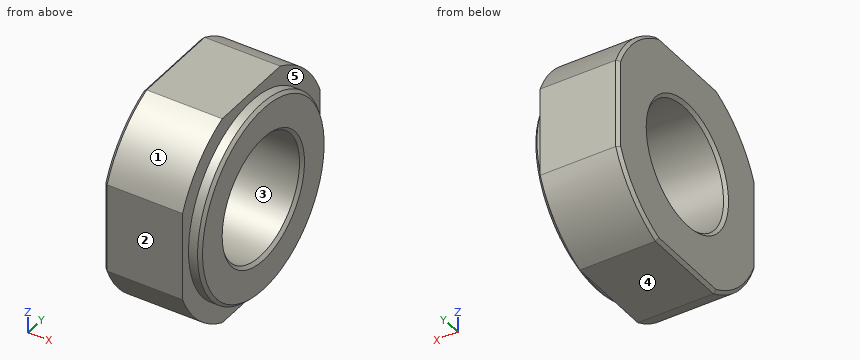
```python
from build123d import *

# Parameters (mm, degrees)
SKETCH1_R           = 19
SKETCH1_R_2         = 10
BOSS_EXTRUDE1_DEPTH = 15
SKETCH2_OUTSIDE_W   = 51.158
SKETCH2_OUTSIDE_H   = 51.158
SKETCH2_OUTSIDE_R   = 16
CUT_EXTRUDE1_DEPTH  = 2
SKETCH3_OUTSIDE_W   = 51.158
SKETCH3_OUTSIDE_H   = 51.158
SKETCH3_OUTSIDE_W_2 = 35
SKETCH3_OUTSIDE_H_2 = 35
CUT_EXTRUDE2_DEPTH  = 31.773365107
CHAMFER1_SIZE       = 0.5


with BuildPart() as part:
    # Sketch1 → Boss-Extrude1 (new body)
    with BuildSketch(Plane(origin=(0, 0, 0), x_dir=(0, 0, -1), z_dir=(1, 0, 0))):
        Circle(SKETCH1_R)
        Circle(SKETCH1_R_2, mode=Mode.SUBTRACT)
    extrude(amount=BOSS_EXTRUDE1_DEPTH)

    # Sketch2 outside → Cut-Extrude1 (cut)
    with BuildSketch(Plane(origin=(15, 0, 0), x_dir=(0, 0, -1), z_dir=(1, 0, 0))):
        Rectangle(SKETCH2_OUTSIDE_W, SKETCH2_OUTSIDE_H)
        Circle(SKETCH2_OUTSIDE_R, mode=Mode.SUBTRACT)
    extrude(amount=-CUT_EXTRUDE1_DEPTH, mode=Mode.SUBTRACT)

    # Sketch3 outside → Cut-Extrude2 (cut, through all)
    with BuildSketch(Plane.ZY):
        Rectangle(SKETCH3_OUTSIDE_W, SKETCH3_OUTSIDE_H)
        Rectangle(SKETCH3_OUTSIDE_W_2, SKETCH3_OUTSIDE_H_2, mode=Mode.SUBTRACT)
    extrude(amount=-CUT_EXTRUDE2_DEPTH, mode=Mode.SUBTRACT)

    # Chamfer1
    chamfer1_edges = [part.edges().sort_by_distance(p)[0] for p in [
        (15, 0, 16),
        (0, 13.435028843, -13.435028843),
        (0, 13.435028843, 13.435028843),
        (0, -13.435028843, 13.435028843),
        (0, -13.435028843, -13.435028843),
        (0, 0, 17.5),
        (0, -17.5, 0),
        (0, 0, -17.5),
        (0, 17.5, 0),
        (0, 0, 10),
        (15, 0, 10),
    ]]
    chamfer(chamfer1_edges, length=CHAMFER1_SIZE)


solid = part.part
```
Source: CAD feature listing. Evaluate the final solid. Frame: model axes, mm. Face numbers are marked on the shaded views. A direction names the side the tool comes from. Round coordinates to 2 decimals unless told otherwise and drop trailing zeros. Order: outer loops, then holes, each group sorted by start corner. A loop starts at its lowest first (then second) coordinate and runs counter-clockwise, first axis right, second up. Notation, with made-up numbers: (24.5, 43.25) -> (40.5, 43.25) arc R12 cw to (40.5, 58.25) -> close; hole circle Ø9 at (79, 44). An arc over 180 degrees is marked (long way). One line per item, written item: value. Start each with the question number.
Q1. Section query A-A (y = 0). Return the cut outline in (x, z), plus the area to 3 significant figures.
Q2. Pin query (flat end, axial travel): pin 1 (4 mm diameter, centred on x = 6, z = 11.5, fed in from -Y); pin 2 (4 mm diameter, centred on x = 3.5, y = 10.5, fed in from +Z); pin 3 (5 mm diameter, centred on y = 0, z = 12, fed in from -X); pin 4 (1.5 mm diameter, centred on x = 3, y = -10, fed in from -Z). Return the tip coordinate at first contact, or that it passes through.
Q3. Section query C-C (x = 1). Return the cut outline in (y, z).
Q4. Access query for the marked faces 4 and 5. Directions: +Z, -Z, +X, -X, +Y, -Y. A direction counts if a zero-diameter tool reaches every point of the face in a straight line with its end or side. Return the directions, or none.
Q5. Material intervals for probe 1 along Y at (x, z) = (4, 0); probe 2 along X at (y, z) = (-16, 3.5); probe 3 along Z at (x, y) = (5, -11), sorted ascending.
Q6. Draft query along Z for the marked faces 1, 2 and 3. Return one class per face: pulls with the +Z half, pulls with the -Z half, needs draft (parallel to the pull), parting line crosses it, or undercut.
Findings below:
1. outline: (0, -17) -> (0.5, -17.5) -> (13, -17.5) -> (13, -16) -> (14.5, -16) -> (15, -15.5) -> (15, -10.5) -> (14.5, -10) -> (0.5, -10) -> (0, -10.5) -> close; (0, 10.5) -> (0.5, 10) -> (14.5, 10) -> (15, 10.5) -> (15, 15.5) -> (14.5, 16) -> (13, 16) -> (13, 17.5) -> (0.5, 17.5) -> (0, 17) -> close
1. area: 218 mm²
2. pin 1: y = -16.45
2. pin 2: z = 16.99
2. pin 3: x = 0
2. pin 4: z = -16.6
3. outline: (-17.5, -7.4) arc R19 ccw to (-7.4, -17.5) -> (7.4, -17.5) arc R19 ccw to (17.5, -7.4) -> (17.5, 7.4) arc R19 ccw to (7.4, 17.5) -> (-7.4, 17.5) arc R19 ccw to (-17.5, 7.4) -> close; hole circle Ø20 at (0, 0)
4. face 4: -Z, +X, -X, +Y, -Y
4. face 5: +X
5. probe 1: -17.5 to -10, 10 to 17.5
5. probe 2: 0 to 13
5. probe 3: -15.49 to 15.49
6. face 1: pulls with the +Z half
6. face 2: needs draft
6. face 3: undercut
